Source: CAD feature listing. Evaluate the final solid. Frame: model axes, mm. A direction names the side the tool comes from. Give positions to 0.01 mm unless a question says otherwise; leave off trailing zeros. Loops run counter-clockwise (first coordinate to the right, second up) from the corner with the lowest first, then second, coordinate; pieces in that order, holes last. Notation, with made-up numbers: (-11, 34) -> (8, 34) arc R32 ccw to (8, 65) -> close; hole circle Ø5 at (1.5, 45.5). An arc over 180 degrees is marked (long way). Return JSON: item names as keys, results as strings. Group by question number.
(1) Ray query, line 1 (Y direction, x = 0, z = -0.25); line 2 (Y direction, x = 6, z = -5.25); line 3 (Z direction, x = 4.25, y = -1). Return the intervals inside material, ascending. Write a range as from..to.
(2) Access query for faces 4 (the face through (-2, 2.5, 2.4)), 5 (the face through (2.5, 0, 3)), 6 (the face through (2, -2.5, 2.6)), 7 (the face through (2, 2.5, 2.4)). Directions: +Z, -Z, +X, -X, +Y, -Y. A direction counts if a zero-diameter tool reaches every point of the face in a straight line with its end or side. Return the directions, or none.
(3) Cut plane B-B on y = 0. Return loops of the section in (x, z), then the cut area to 3 significant figures.
(4) Pin query (flat end, axial travel): pin 1 (2 mm diameter, centred on y = -0.5, z = 0.5, fed in from +X); pin 2 (1.8 mm diameter, centred on x = -5, y = 1, fed in from +Z). Return the tip coordinate at first contact, or that it passes through.
(5) Cut plane A-A on x = 6. Return loops of the section in (y, z), then the cut area to 3 significant figures.
(6) Draft query along Y for faces 1 (the face through (-1.216, 1.115, 0.105)), 2 (the face through (8.5, -2.5, -5)), 3 (the face through (-2, 0, -7.5)). Return one class per face: released by +Y, released by -Y, zero draft, split by the parting line, or undercut.
(7) Cut plane C-C on z = -4.75. Return loops of the section in (x, y).
(8) Cut plane D-D on z = 3.75. Return loops of the section in (x, y), then the cut area to 3 significant figures.
```python
from build123d import *

# Parameters (mm, degrees)
SKETCH3_W            = 18
SKETCH3_H            = 15
BOSS_EXTRUDE2_DEPTH  = 3
M3_CLEARANCE_HOLE1_D = 3.4
CHAMFER1_SIZE        = 1
SKETCH10_W           = 6.5
SKETCH10_H           = 10
CUT_EXTRUDE1_DEPTH   = 14.162446581
M4_TAPPED_HOLE1_D    = 3.3
CHAMFER2_SIZE        = 1


with BuildPart() as part:
    # Sketch3 → Boss-Extrude2 (new, symmetric)
    with BuildSketch(Plane(origin=(0, 0, 0), x_dir=(1, 0, 0), z_dir=(0, 1, 0))):
        Rectangle(SKETCH3_W, SKETCH3_H)
    extrude(amount=BOSS_EXTRUDE2_DEPTH, both=True)

    # M3 Clearance Hole1 (through all)
    with Locations(Plane(origin=(0, 0, -7.5), x_dir=(-1, 0, 0), z_dir=(0, 0, -1))):
        with Locations((-6, 0), (6, 0)):
            Hole(M3_CLEARANCE_HOLE1_D / 2)

    # Chamfer1
    chamfer1_edges = [part.edges().sort_by_distance(p)[0] for p in [
        (-9, 3, 0),
        (-9, -3, 0),
        (9, -3, 0),
        (9, 3, 0),
    ]]
    chamfer(chamfer1_edges, length=CHAMFER1_SIZE)

    # Sketch10 → Cut-Extrude1 (cut, through all)
    with BuildSketch(Plane(origin=(0, -3, 0), x_dir=(-1, 0, 0), z_dir=(0, -1, 0))):
        with Locations((-5.75, -2.5)):
            Rectangle(SKETCH10_W, SKETCH10_H)
        with Locations((5.75, -2.5)):
            Rectangle(SKETCH10_W, SKETCH10_H)
    extrude(amount=-CUT_EXTRUDE1_DEPTH, mode=Mode.SUBTRACT)

    # M4 Tapped Hole1 (through all)
    with Locations(Plane(origin=(0, 0, -7.5), x_dir=(-1, 0, 0), z_dir=(0, 0, -1))):
        with Locations((0, 0)):
            Hole(M4_TAPPED_HOLE1_D / 2)

    # Chamfer2
    chamfer2_edges = [part.edges().sort_by_distance(p)[0] for p in [
        (2.5, 3, 2.5),
        (2.5, -3, 2.5),
        (-2.5, 3, 2.5),
        (-2.5, -3, 2.5),
    ]]
    chamfer(chamfer2_edges, length=CHAMFER2_SIZE)


solid = part.part
```
Answers:
{
 "1": {"line 1": "-3..-1.65, 1.65..3", "line 2": "-3..-1.7, 1.7..3", "line 3": "-7.5..-2.5"},
 "2": {"face 4": "+Z, -X, +Y", "face 5": "+Z, +X, +Y, -Y", "face 6": "+Z, +X, -Y", "face 7": "+Z, +X, +Y"},
 "3": {"outline": "(-9, -7.5) -> (-7.7, -7.5) -> (-7.7, -2.5) -> (-9, -2.5) -> close; (-4.3, -7.5) -> (-1.65, -7.5) -> (-1.65, 7.5) -> (-2.5, 7.5) -> (-2.5, -2.5) -> (-4.3, -2.5) -> close; (1.65, -7.5) -> (4.3, -7.5) -> (4.3, -2.5) -> (2.5, -2.5) -> (2.5, 7.5) -> (1.65, 7.5) -> close; (7.7, -7.5) -> (9, -7.5) -> (9, -2.5) -> (7.7, -2.5) -> close", "area": "56.5 mm²"},
 "4": {"pin 1": "x = 2.5", "pin 2": "z = -2.5"},
 "5": {"outline": "(-3, -7.5) -> (-1.7, -7.5) -> (-1.7, -2.5) -> (-3, -2.5) -> close; (1.7, -7.5) -> (3, -7.5) -> (3, -2.5) -> (1.7, -2.5) -> close", "area": "13.0 mm²"},
 "6": {"face 1": "undercut", "face 2": "released by -Y", "face 3": "zero draft"},
 "7": {"outline": "(-9, -2) -> (-8, -3) -> (8, -3) -> (9, -2) -> (9, 2) -> (8, 3) -> (-8, 3) -> (-9, 2) -> close; hole circle Ø3.4 at (-6, 0); hole circle Ø3.3 at (0, 0); hole circle Ø3.4 at (6, 0)"},
 "8": {"outline": "(-2.5, -2) -> (-1.5, -3) -> (1.5, -3) -> (2.5, -2) -> (2.5, 2) -> (1.5, 3) -> (-1.5, 3) -> (-2.5, 2) -> close; hole circle Ø3.3 at (0, 0)", "area": "19.4 mm²"}
}
